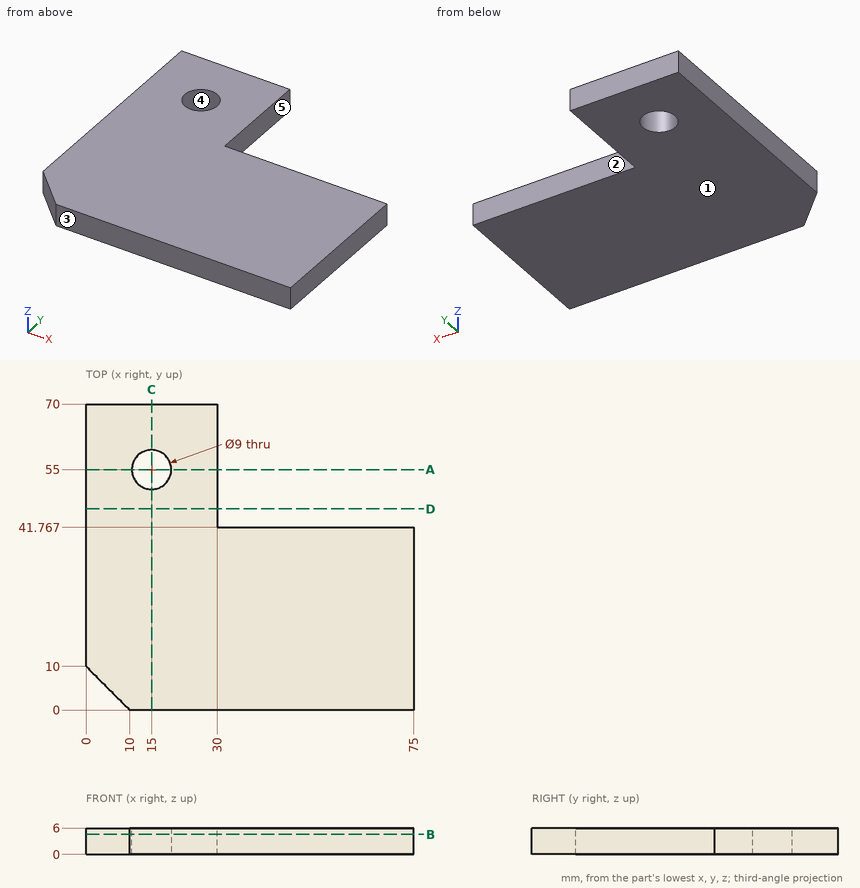
Can you work these out from the drawing? Everything is in mm from the part's minimum corner. A direction names the side the tool comes from. Coordinates: 2 decimals unless noted, no trailing zeros. Loops run counter-clockwise (first coordinate to the right, second up) from the corner with the lowest first, then second, coordinate; pieces in that order, holes last. Notation, with made-up numbers: (21.25, -31.5) - (52.25, -31.5) arc R25 cw to (52.25, -0.5) - close; hole circle Ø11 at (-5.5, 30). An arc over 180 degrees is marked (long way). Put each result on its own line as item: value. Start each with the question number.
Item 1: If we mould it in two halves opening along X, with no side actions, what happens to the marked faces 3, 4 and 5? For each: +X half, -X half, draft (parallel to the pull), parting line (faces both ways), or undercut.
Item 2: For pin 1 (8 mm diameter, centred on x = 15, y = 55, fed in from -Z); pin 2 (1 mm diameter, centred on y = 51, z = 3.5, fed in from +X), each with a flat end and sliding along its axis, tell me the tip position at first contact or that it passes through.
Item 3: If I drill on line 1 along Y through (x, z) = (15, 4.5); line 2 along X through (y, z) = (46, 1.65); line 3 along Y through (x, z) = (65.5, 1.9), over which ranges is the centre line in solid material (lowest first)?
Item 4: Which directions (+Z, -Z, +X, -X, +Y, -Y) give clear straight access to the entire face, cutting with the end or side of a thin tool? Please do the marked faces 1 and 2.
Item 5: Suppose I cut it at D-D (y = 46). Please give me the cut outline in (x, z), and give its area (3 significant figures).
Item 6: Suppose I cut it at B-B (z = 4.55). Please give me the cut outline in (x, y), and give its area (3 significant figures).
Item 7: Suppose I cut it at C-C (x = 15). Please give me the cut outline in (y, z).
Item 8: Suppose I cut it at A-A (y = 55). Please give me the cut outline in (x, z), and give its area (3 significant figures).
Here are the results:
1. face 3: draft
1. face 4: undercut
1. face 5: +X half
2. pin 1: through
2. pin 2: x = 30
3. line 1: 0 to 50.5, 59.5 to 70
3. line 2: 0 to 30
3. line 3: 0 to 41.77
4. face 1: -Z, +X, -X, +Y, -Y
4. face 2: +Z, -Z, +X, +Y
5. outline: (0, 0) - (30, 0) - (30, 6) - (0, 6) - close
5. area: 180 mm²
6. outline: (0, 10) - (10, 0) - (75, 0) - (75, 41.77) - (30, 41.77) - (30, 70) - (0, 70) - close; hole circle Ø9 at (15, 55)
6. area: 3,870 mm²
7. outline: (0, 0) - (50.5, 0) - (50.5, 6) - (0, 6) - close; (59.5, 0) - (70, 0) - (70, 6) - (59.5, 6) - close
8. outline: (0, 0) - (10.5, 0) - (10.5, 6) - (0, 6) - close; (19.5, 0) - (30, 0) - (30, 6) - (19.5, 6) - close
8. area: 126 mm²
